Can you work these out from the drawing? Everything is in mm from the part's minimum corner. A direction names the side the tool comes from. Round coordinates to 2 decimals unless told otherwise and drop trailing zeros. Order: outer loops, then holes, each group sorted by start corner. A loop starts at its lowest first (then second) coordinate and runs counter-clockwise, first axis right, second up. Notation, with made-up numbers: (9.5, -32.5) - (17.5, -32.5) arc R24 cw to (17.5, -7.5) - close; hole circle Ø8 at (62.5, 75.5). An arc over 180 degrees is marked (long way). Write item = value, one per line.
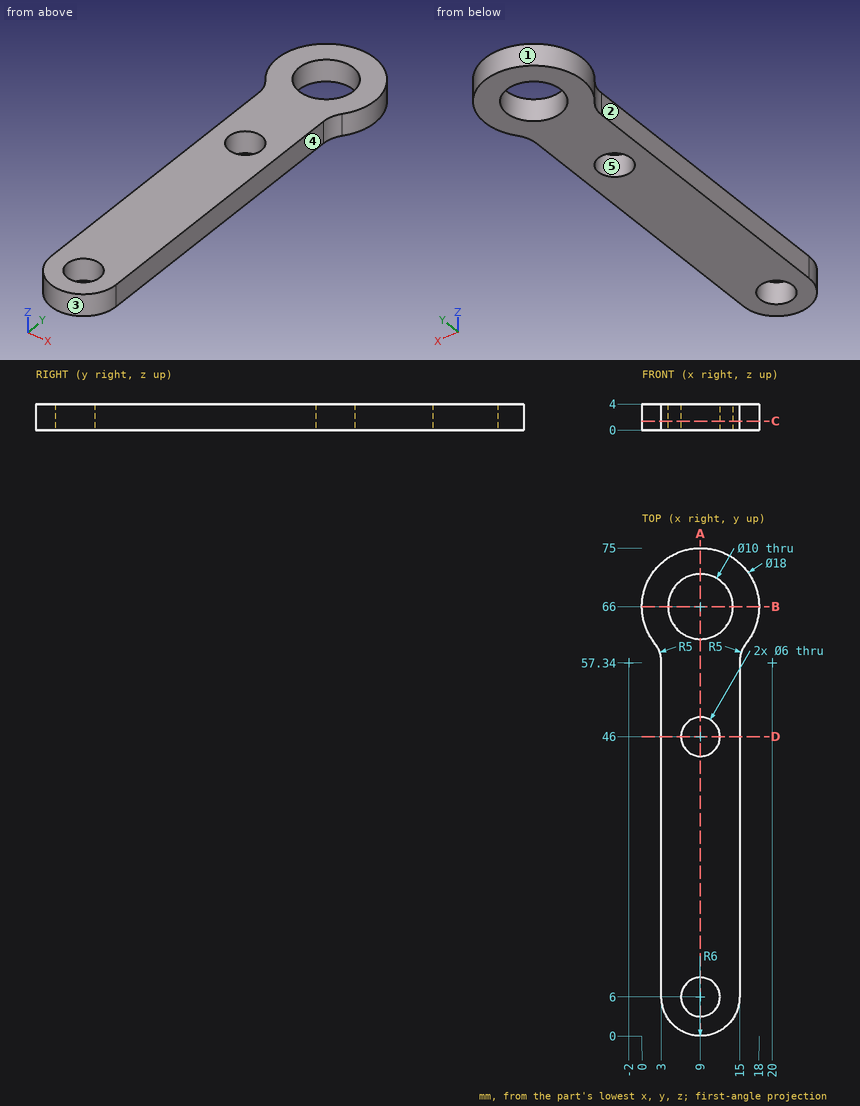
(1) Thinking about a two-plate mould opening in X: for the marked faces 3, 4 and 5, which applies, +X half, -X half, draft (parallel to the pull), parting line (faces both ways), or undercut?
Computed:
face_3 = parting line
face_4 = +X half
face_5 = undercut
(2) If we section it at D-D (y = 46): Write out the boundary of the cut face in (x, z), plus the area to 3 significant figures.
Computed:
outline = (3, 0) - (6, 0) - (6, 4) - (3, 4) - close; (12, 0) - (15, 0) - (15, 4) - (12, 4) - close
area = 24.0 mm^2
(3) If I drill on line 1 (Y direction, x = 9, z = 2.5); line 2 (X direction, y = 29, z = 1.2); line 3 (Y direction, x = 10.25, z = 3.2), over which ranges is the centre line in solid material (lowest first)? Write a range as from..to.
Computed:
line_1 = 0..3, 9..43, 49..61, 71..75
line_2 = 3..15
line_3 = 0.13..3.27, 8.73..43.27, 48.73..61.16, 70.84..74.91
(4) If we section it at A-A (x = 9): Write out the boundary of the cut face in (y, z).
Computed:
outline = (0, 0) - (3, 0) - (3, 4) - (0, 4) - close; (9, 0) - (43, 0) - (43, 4) - (9, 4) - close; (49, 0) - (61, 0) - (61, 4) - (49, 4) - close; (71, 0) - (75, 0) - (75, 4) - (71, 4) - close
(5) If we section it at B-B (y = 66): Write out the boundary of the cut face in (x, z).
Computed:
outline = (0, 0) - (4, 0) - (4, 4) - (0, 4) - close; (14, 0) - (18, 0) - (18, 4) - (14, 4) - close
(6) On a 3-axis mill with a long thin cutter (end or side, diameter ignored), from which of +Z, -Z, +X, -X, +Y, -Y can I reach the whole of each face in a straight line? I mean the marked faces 1 and 2. Say none if no direction works.
Computed:
face_1 = +Z, -Z
face_2 = +Z, -Z, -X, -Y
(7) Will these pins go through, and if not, where does the flat tip stop? P1, Ø2, axis at y = 28.5, z = 0.5, coming from the +X side; P2, Ø8, axis at x = 9, y = 46, coming from the -Z side.
Computed:
P1 = 15
P2 = 0
(8) If we section it at C-C (z = 1.35): Write out the boundary of the cut face in (x, y).
Computed:
outline = (1.93, 60.43) arc R5 cw to (3, 57.34) - (3, 6) arc R6 ccw to (15, 6) - (15, 57.34) arc R5 cw to (16.07, 60.43) arc R9 ccw (long way) to start; hole circle Ø10 at (9, 66); hole circle Ø6 at (9, 6); hole circle Ø6 at (9, 46)
